```python
from build123d import *

# Parameters (mm, degrees)
SKETCH1_R           = 30
BOSS_EXTRUDE1_DEPTH = 20
SKETCH2_R           = 29.5
BOSS_EXTRUDE2_DEPTH = 45
SKETCH3_R           = 30
BOSS_EXTRUDE3_DEPTH = 15
SKETCH4_R           = 8
CUT_EXTRUDE1_DEPTH  = 65
SKETCH5_R           = 11.25
BOSS_EXTRUDE4_DEPTH = 10
FILLET1_R           = 10
SKETCH6_R           = 4.25
CUT_EXTRUDE2_DEPTH  = 90.101417022
SKETCH_7_2_R        = 8
CUT_EXTRUDE3_DEPTH  = 1
CUT_EXTRUDE4_REACH  = 91.101
SKETCH_7_2_2_R      = 8


with BuildPart() as part:
    # Sketch1 → Boss-Extrude1 (new body)
    with BuildSketch(Plane.XY):
        Circle(SKETCH1_R)
    extrude(amount=-BOSS_EXTRUDE1_DEPTH)

    # Sketch2 → Boss-Extrude2 (add)
    with BuildSketch(Plane(origin=(0, 0, -20), x_dir=(-1, 0, 0), z_dir=(0, 0, -1))):
        with Locations(Location((0, 0, 0), (0, 0, 180))):
            Circle(SKETCH2_R)
    extrude(amount=BOSS_EXTRUDE2_DEPTH)

    # Sketch3 → Boss-Extrude3 (add)
    with BuildSketch(Plane(origin=(0, 0, -65), x_dir=(-1, 0, 0), z_dir=(0, 0, -1))):
        with Locations(Location((0, 0, 0), (0, 0, 180))):
            Circle(SKETCH3_R)
    extrude(amount=BOSS_EXTRUDE3_DEPTH)

    # Sketch4 → Cut-Extrude1 (cut)
    with BuildSketch(Plane.XY):
        Circle(SKETCH4_R)
    extrude(amount=-CUT_EXTRUDE1_DEPTH, mode=Mode.SUBTRACT)

    # Sketch5 → Boss-Extrude4 (add)
    with BuildSketch(Plane.XY):
        with Locations((35, 0)):
            Circle(SKETCH5_R)
        with Locations((-35, 0)):
            Circle(SKETCH5_R)
    extrude(amount=-BOSS_EXTRUDE4_DEPTH)

    # Fillet1
    fillet1_edges = [part.edges().sort_by_distance(p)[0] for p in [
        (28.549107143, 9.216750042, -5),
        (28.549107143, -9.216750042, -5),
        (-28.549107143, -9.216750042, -5),
        (-28.549107143, 9.216750042, -5),
    ]]
    fillet(fillet1_edges, radius=FILLET1_R)

    # Sketch6 → Cut-Extrude2 (cut, through all)
    with BuildSketch(Plane(origin=(0, 0, -10), x_dir=(-1, 0, 0), z_dir=(0, 0, -1))):
        with Locations((37.5, 0)):
            Circle(SKETCH6_R)
        with Locations((-37.5, 0)):
            Circle(SKETCH6_R)
    extrude(amount=-CUT_EXTRUDE2_DEPTH, mode=Mode.SUBTRACT)

    # Sketch 7_2 → Cut-Extrude3 (cut)
    with BuildSketch(Plane(origin=(0, 0, -10), x_dir=(-1, 0, 0), z_dir=(0, 0, -1))):
        with Locations((37.5, 0)):
            Circle(SKETCH_7_2_R)
        with Locations((-37.5, 0)):
            Circle(SKETCH_7_2_R)
    extrude(amount=-CUT_EXTRUDE3_DEPTH, mode=Mode.SUBTRACT)

    # Sketch 7_2 2 → Cut-Extrude4 (cut, up to next)
    with BuildSketch(Plane(origin=(0, 0, -10), x_dir=(-1, 0, 0), z_dir=(0, 0, -1)), mode=Mode.PRIVATE) as cut_extrude4_sk1:
        with Locations((37.5, 0)):
            Circle(SKETCH_7_2_2_R)
    cut_extrude4_tool1 = extrude(cut_extrude4_sk1.sketch, amount=CUT_EXTRUDE4_REACH, mode=Mode.PRIVATE) & part.part
    # Sketch 7_2 2 → Cut-Extrude4 (cut, up to next)
    with BuildSketch(Plane(origin=(0, 0, -10), x_dir=(-1, 0, 0), z_dir=(0, 0, -1)), mode=Mode.PRIVATE) as cut_extrude4_sk2:
        with Locations((-37.5, 0)):
            Circle(SKETCH_7_2_2_R)
    cut_extrude4_tool2 = extrude(cut_extrude4_sk2.sketch, amount=CUT_EXTRUDE4_REACH, mode=Mode.PRIVATE) & part.part
    add(cut_extrude4_tool1.solids().sort_by_distance((-37.5, 0, -10))[0], mode=Mode.SUBTRACT)
    add(cut_extrude4_tool2.solids().sort_by_distance((37.5, 0, -10))[0], mode=Mode.SUBTRACT)


solid = part.part
```
Geometry: final body of the model. Coordinates: model frame, mm. A direction names the side the tool comes from. Coordinates: 2 decimals unless noted, no trailing zeros. Loops run counter-clockwise (first coordinate to the right, second up) from the corner with the lowest first, then second, coordinate; pieces in that order, holes last. Notation, with made-up numbers: (85, 9) -> (131, 9) arc R24 ccw to (131, 27) -> close; hole circle Ø3 at (-12, 27). An arc over 180 degrees is marked (long way). Use a Markdown table: item, result. Add a question column.
(1) Section query A-A, the plane z = -18.5. Return loops of the section in (x, y), plus the area to 3 significant figures.
(2) Section query D-D, the plane y = 9.5. Return loops of the section in (x, z), plus the area to 3 significant figures.
(3) Pin query (flat end, axial travel): pin 1 Ø12 at (y, z) = (-8.5, -28) entering from -X; pin 2 Ø8 at (x, y) = (1, 3.5) entering from +Z; pin 3 Ø8 at (x, y) = (40, -0.5) entering from -Z. Return the tip coordinate at first contact, or that it passes through.
(4) Section query B-B, the plane x = 38.5. Return loops of the section in (y, z).
(5) Line query: line 1 along Z through (x, y) = (-20.5, 21.5); line 2 along Z through (x, y) = (-35, -7); line 3 along Y through (x, z) = (37.5, -5.25). Output: solid intervals per line, ascending.
(6) Access query for faces 5 (the cylindrical face through (0.625, 29.993, -9.86)), 6 (the flat face through (-4.6, -29.4, -20)), 7 (the flat face through (0, 0, -65)), 8 (the cylindrical face through (29.517, -0.526, -13.303)), 9 (the cylindrical face through (-0.625, -29.993, -9.86)). Directions: +Z, -Z, +X, -X, +Y, -Y. A direction counts if a zero-diameter tool reaches every point of the face in a straight line with its end or side. Return the directions, or none.
(7) Section query C-C, the plane x = 2.5. Return loops of the section in (y, z).
(8) Mould query, pull axis Z, two halves, no side actions, for faces 1 (the cylindrical face through (28.14, -8.86, -42.18)), 2 (the cylindrical face through (-33.254, 0.187, -4.563)), 3 (the flat face through (-30, -5, -10)), 4 (the flat face through (22, 20, -65)). Classes: pulls with the +Z half, pulls with the -Z half, needs draft (parallel to the pull), parting line crosses it, or undercut.
Answer:
| question | item | result |
|---|---|---|
| 1 | outline | (-29.9, -2.49) arc R30 ccw to (29.9, -2.49) arc R8 cw to (29.9, 2.49) arc R30 ccw to (-29.9, 2.49) arc R8 cw to start; hole circle Ø16 at (0, 0) |
| 1 | area | 2,620 mm^2 |
| 2 | outline | (-41.03, -10) -> (-28.46, -10) -> (-28.46, -20) -> (-27.93, -20) -> (-27.93, -65) -> (-28.46, -65) -> (-28.46, -80) -> (28.46, -80) -> (28.46, -65) -> (27.93, -65) -> (27.93, -20) -> (28.46, -20) -> (28.46, -10) -> (41.03, -10) -> (41.03, 0) -> (-41.03, 0) -> close |
| 2 | area | 4,760 mm^2 |
| 3 | pin 1 | stops at x = -29.39 |
| 3 | pin 2 | stops at z = -65 |
| 3 | pin 3 | stops at z = -9 |
| 4 | outline | (-10.69, -10) -> (-7.94, -10) -> (-7.94, -9) -> (-4.13, -9) -> (-4.13, 0) -> (-10.69, 0) -> close; (4.13, -9) -> (7.94, -9) -> (7.94, -10) -> (10.69, -10) -> (10.69, 0) -> (4.13, 0) -> close |
| 5 | line 1 | z = -80 to -65, -20 to 0 |
| 5 | line 2 | z = -9 to 0 |
| 5 | line 3 | y = -10.97 to -4.25, 4.25 to 10.97 |
| 6 | face 5 | -Z, +Y |
| 6 | face 6 | -Y |
| 6 | face 7 | +Z |
| 6 | face 8 | none |
| 6 | face 9 | -Z, -Y |
| 7 | outline | (-29.9, -80) -> (29.9, -80) -> (29.9, -65) -> (29.39, -65) -> (29.39, -20) -> (29.9, -20) -> (29.9, 0) -> (7.6, 0) -> (7.6, -65) -> (-7.6, -65) -> (-7.6, 0) -> (-29.9, 0) -> (-29.9, -20) -> (-29.39, -20) -> (-29.39, -65) -> (-29.9, -65) -> close |
| 8 | face 1 | undercut |
| 8 | face 2 | needs draft |
| 8 | face 3 | pulls with the -Z half |
| 8 | face 4 | undercut |
